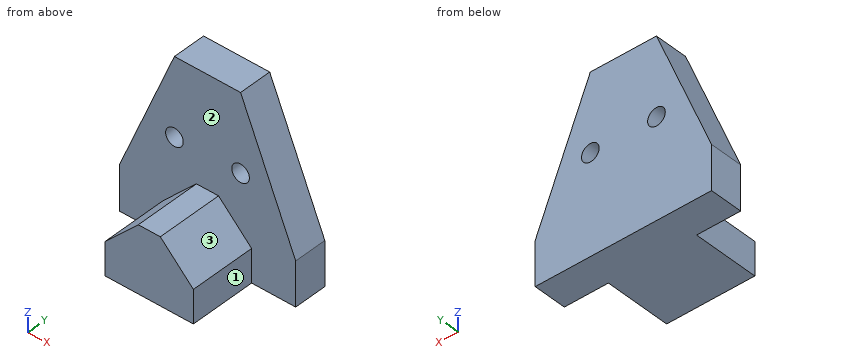
from build123d import *

# Parameters (mm, degrees)
BASE_PLATE_SKETCH_W      = 80
BASE_PLATE_SKETCH_H      = 10
BASE_PLATE_DEPTH         = 20
PENTAGONAL_BOSS_DEPTH    = 15
FOUR_SIDED_BOSS_SKETCH_W = 80
FOUR_SIDED_BOSS_SKETCH_H = 5
FOUR_SIDED_BOSS_DEPTH    = 20
OCTAGONAL_BOSS_DEPTH     = 30
HOLES_2X_8_SKETCH_R      = 4
HOLES_2X_8_DEPTH         = 15


with BuildPart() as part:
    # Base Plate Sketch → Base Plate (new body)
    with BuildSketch(Plane.XY):
        with Locations((40, 5)):
            Rectangle(BASE_PLATE_SKETCH_W, BASE_PLATE_SKETCH_H)
    extrude(amount=BASE_PLATE_DEPTH)

    # Pentagonal Boss Sketch → Pentagonal Boss (add)
    with BuildSketch(Plane.XZ):
        Polygon((40, 80), (25, 80), (0, 20), (80, 20), (55, 80), align=None)
    extrude(amount=-PENTAGONAL_BOSS_DEPTH)

    # Four-Sided Boss Sketch → Four-Sided Boss (add)
    with BuildSketch(Plane(origin=(0, 0, 0), x_dir=(-1, 0, 0), z_dir=(0, 0, -1))):
        with Locations((-40, 12.5)):
            Rectangle(FOUR_SIDED_BOSS_SKETCH_W, FOUR_SIDED_BOSS_SKETCH_H)
    extrude(amount=-FOUR_SIDED_BOSS_DEPTH)

    # Octagonal Boss Sketch → Octagonal Boss (add)
    with BuildSketch(Plane.XZ):
        Polygon((40, 0), (60, 0), (60, 15), (45, 30), (40, 30), (35, 30), (20, 15), (20, 0), align=None)
    extrude(amount=OCTAGONAL_BOSS_DEPTH)

    # Holes 2xØ8 Sketch → Holes 2xØ8 (cut)
    with BuildSketch(Plane.XZ):
        with Locations(Location((25, 45, 0), (0, 0, 270))):
            Circle(HOLES_2X_8_SKETCH_R)
        with Locations(Location((55, 45, 0), (0, 0, 270))):
            Circle(HOLES_2X_8_SKETCH_R)
    extrude(amount=-HOLES_2X_8_DEPTH, mode=Mode.SUBTRACT)


solid = part.part
For this review, take the finished solid that the model builds, in its own axes (mm). Face numbers are marked on the shaded views. A direction names the side the tool comes from. Give positions to 0.01 mm unless a question says otherwise; leave off trailing zeros. Loops run counter-clockwise (first coordinate to the right, second up) from the corner with the lowest first, then second, coordinate; pieces in that order, holes last.
Item 1: Insertion check: pin 1 (16.5 mm diameter, centred on y = -9, z = 11, fed in from +X); pin 2 (4.5 mm diameter, centred on y = -16.5, z = 11, fed in from -X); pin 3 (12 mm diameter, centred on x = 33, y = 10.5, fed in from -Z); pin 4 (3 mm diameter, centred on x = 39.5, y = -14.5, fed in from +Z). Each pin has a flat end and moves straight along its axis. Give the tip position at first contact, or say it passes through.
Item 2: Take a section at B-B, the plane y = -24.5. State the section outline as (x, z) points.
Item 3: Take a section at A-A, the plane z = 45. State the section outline as (x, y) points, and give its area (4 significant figures).
Item 4: Take a section at D-D, the plane z = 12. State the section outline as (x, y) points.
Item 5: Take a section at C-C, the plane x = 42. State the section outline as (y, z) points.
Item 6: For line 1 along X through (y, z) = (4.25, 45); line 2 along X through (y, z) = (-1, 10); line 3 along Y through (x, z) = (18, 8), list the stretches that pass through material, from the lowest coordinate up.
Item 7: Tool access review of the marked faces 1, 2 and 3: name each direction out of +Z, -Z, +X, -X, +Y, -Y from which nothing blocks a thin tool from reaching the whole face with its end or side.
Calculated:
1. pin 1: stops at x = 60
1. pin 2: stops at x = 20
1. pin 3: stops at z = 0
1. pin 4: stops at z = 30
2. outline: (20, 0) - (60, 0) - (60, 15) - (45, 30) - (35, 30) - (20, 15) - close
3. outline: (10.42, 0) - (21, 0) - (21, 15) - (10.42, 15) - close; (29, 0) - (51, 0) - (51, 15) - (29, 15) - close; (59, 0) - (69.58, 0) - (69.58, 15) - (59, 15) - close
3. area: 647.5 mm2
4. outline: (0, 0) - (20, 0) - (20, -30) - (60, -30) - (60, 0) - (80, 0) - (80, 15) - (0, 15) - close
5. outline: (-30, 0) - (15, 0) - (15, 80) - (0, 80) - (0, 30) - (-30, 30) - close
6. line 1: x = 10.42 to 21, 29 to 51, 59 to 69.58
6. line 2: x = 20 to 60
6. line 3: y = 0 to 15
7. face 1: +Z, -Z, +X, -Y
7. face 2: +Z, -Y
7. face 3: +Z, +X, -Y
